The model under review builds one solid part; all positions refer to its coordinate system, in mm. A direction names the side the tool comes from. Round coordinates to 2 decimals unless told otherwise and drop trailing zeros. Loops run counter-clockwise (first coordinate to the right, second up) from the corner with the lowest first, then second, coordinate; pieces in that order, holes last. Notation, with made-up numbers: (-16.75, 10.5) -> (42.25, 10.5) arc R19 cw to (42.25, 40.5) -> close; hole circle Ø5 at (-13, 1). An arc over 180 degrees is marked (long way). Use a Markdown table: item, result. Add a question column.
1) Insertion check: pin 1 (6 mm diameter, centred on y = 2, z = -2, fed in from +X); pin 2 (4 mm diameter, centred on y = 6.5, z = -1.5, fed in from -X); pin 3 (3 mm diameter, centred on x = 9.5, z = -2.5, fed in from +Y). Each pin has a flat end and moves straight along its axis. Give the tip position at first contact, or say it passes through.
2) For faces 1 (the flat face through (0, 0, 0)), 2 (the flat face through (-11, -7, -7)), list the 3-axis set-ups (+Z, -Z, +X, -X, +Y, -Y) from which the entire face can be reached by the end or side of a thin tool; tool diameter is ignored.
3) Wall thickness on probe 1 along Z at (x, y) = (12, -4); probe 2 along X at (y, z) = (4, -3); probe 3 along X at (y, z) = (2.75, -9.5): over which ranges is each line inside the solid? List them lowest first.
4) Consider section C-C on z = -4.25. Give the boundary of the cut face in (x, y), plus the area to 3 significant figures.
5) Consider section A-A on y = 0. Give the boundary of the cut face in (x, z), plus the area to 4 significant figures.
from build123d import *

# Parameters (mm, degrees)
CHAMFER1_SIZE = 1
CHAMFER2_SIZE = 0.5


with BuildPart() as part:
    # Sketch1 → Revolve1 (revolve)
    with BuildSketch(Plane(origin=(0, 0, 0), x_dir=(0, 0, -1), z_dir=(1, 0, 0)), mode=Mode.PRIVATE) as revolve1_sk:
        Polygon((10, 0), (10, 15), (7, 15), (7, 12.5), (0, 12.5), (0, 0), align=None)
    revolve(revolve1_sk.sketch.rotate(Axis((0, 0, 0), (0, 0, -1)), 90), axis=Axis((0, 0, 0), (0, 0, -1)))

    # Chamfer1
    chamfer1_edges = [part.edges().sort_by_distance(p)[0] for p in [
        (-12.5, 0, 0),
    ]]
    chamfer(chamfer1_edges, length=CHAMFER1_SIZE)

    # Chamfer2
    chamfer2_edges = [part.edges().sort_by_distance(p)[0] for p in [
        (-15, 0, -7),
        (-15, 0, -10),
    ]]
    chamfer(chamfer2_edges, length=CHAMFER2_SIZE)


solid = part.part
Result set:
| question | item | result |
|---|---|---|
| 1 | pin 1 | x = 12.5 |
| 1 | pin 2 | x = -11.66 |
| 1 | pin 3 | y = 9.6 |
| 2 | face 1 | +Z, +X, -X, +Y, -Y |
| 2 | face 2 | +Z |
| 3 | probe 1 | -10 to -7 |
| 3 | probe 2 | -11.84 to 11.84 |
| 3 | probe 3 | -14.75 to 14.75 |
| 4 | outline | circle Ø25 at (0, 0) |
| 4 | area | 491 mm2 |
| 5 | outline | (-15, -9.5) -> (-14.5, -10) -> (14.5, -10) -> (15, -9.5) -> (15, -7.5) -> (14.5, -7) -> (12.5, -7) -> (12.5, -1) -> (11.5, 0) -> (-11.5, 0) -> (-12.5, -1) -> (-12.5, -7) -> (-14.5, -7) -> (-15, -7.5) -> close |
| 5 | area | 263.5 mm2 |
